Can you work these out from the model? Positions are in its coordinate system, mm. Face numbers are marked on the shaded views. A direction names the side the tool comes from. Give positions to 0.01 mm unless a question says otherwise; leave off trailing zeros. Loops run counter-clockwise (first coordinate to the right, second up) from the corner with the lowest first, then second, coordinate; pieces in that order, holes last. Notation, with made-up numbers: M -14.5,4.5 L 40.5,4.5 A21 cw 40.5,14.5 Z; hole C -37.5,1 d2. An arc over 180 degrees is marked long. Put each result on its own line as item: value. Start each with the question number.
1) If we mould it in two halves opening along Z, with no side actions, what happens to the marked faces 3, 4 and 5? For each: +Z half, -Z half, draft (parallel to the pull), parting line (faces both ways), or undercut.
2) Imagine slicing it at B-B (x = 0). Write out the boundary of the cut face in (y, z), then the cut area to 3 significant figures.
3) For the marked faces 1 and 2, which set-ups out of +Z, -Z, +X, -X, +Y, -Y let a thin tool reach every point of the face, with its end or its side?
4) For P1, Ø8, axis at y = 16, z = -21, coming from the +X side; P2, Ø2, axis at x = 3, y = -0.5, coming from the +Z side; P3, Ø1.5, axis at y = -3.5, z = 9.5, coming from the -X side; P4, Ø5, axis at y = 17.5, z = 12.5, coming from the -X side, each with a flat end and sliding along its axis, tell me the tip position at first contact or that it passes through.
5) Imagine slicing it at A-A (z = 0). Write out the boundary of the cut face in (x, y).
6) Imagine slicing it at D-D (z = 25.5). Write out the boundary of the cut face in (x, y), then the cut area to 3 significant figures.
7) Please list where these lines run through material, in increasing order: line 1 along X through (y, z) = (8, 0); line 2 along X through (y, z) = (-5, 0.5); line 3 along Y through (x, z) = (-94, 11). Write a range as from..to.
8) Imagine slicing it at C-C (y = -6.5). Write out the boundary of the cut face in (x, z), then the cut area to 3 significant figures.
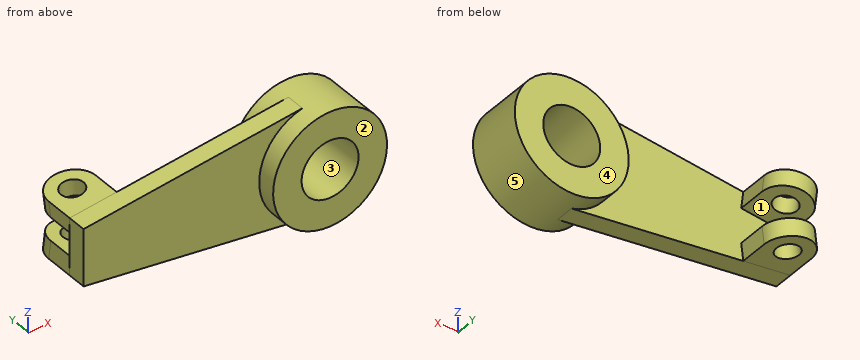
from build123d import *

# Parameters (mm, degrees)
HUB_PROFILE_SKETCH_R   = 30
HUB_60_DEPTH           = 20
LEVER_ARM_DEPTH        = 10
HUB_START              = 20
HUB_EXTENSION_SKETCH_R = 30
HUB_EXTENSION_DEPTH    = 20
CLEVIS_LUG_SKETCH_R    = 6
CLEVIS_LUG_DEPTH       = 9
HUB_RECESS_SKETCH_R    = 30
HUB_RECESS_CUT_DEPTH   = 10
BORE_SKETCH_R          = 15
HUB_BORE_30_DEPTH      = 46


with BuildPart() as part:
    # Hub Profile Sketch → Hub Ø60 (new body)
    with BuildSketch(Plane(origin=(0, 0, 0), x_dir=(1, 0, 0), z_dir=(0, 1, 0))):
        with Locations(Location((0, 0, 0), (0, 0, 270))):
            Circle(HUB_PROFILE_SKETCH_R)
    extrude(amount=HUB_60_DEPTH)

    # Arm Profile Sketch → Lever Arm (add)
    with BuildSketch(Plane(origin=(0, 0, 0), x_dir=(1, 0, 0), z_dir=(0, 1, 0))):
        with BuildLine():
            Line((-122.5, 0), (-30, 0))
            ThreePointArc((-30, 0), (-23.63421499, 18.477658992), (-7.238407879, 29.113664341))
            Line((-7.238407879, 29.113664341), (-122.5, 15))
            Line((-122.5, 15), (-122.5, 0))
        make_face()
        with BuildLine():
            ThreePointArc((-7.238407879, -29.113664341), (-23.63421499, -18.477658992), (-30, 0))
            Line((-30, 0), (-122.5, 0))
            Line((-122.5, 0), (-122.5, -15))
            Line((-122.5, -15), (-7.238407879, -29.113664341))
        make_face()
    extrude(amount=LEVER_ARM_DEPTH)

    # Hub Extension Sketch → Hub Extension (add)
    with BuildSketch(Plane.XZ.offset(HUB_START)):
        with Locations(Location((0, 0, 0), (0, 0, 270))):
            Circle(HUB_EXTENSION_SKETCH_R)
    extrude(amount=-HUB_EXTENSION_DEPTH)

    # Clevis Lug Sketch → Clevis Lug (add)
    with BuildSketch(Plane(origin=(-3.619203939, 0, -29.556832171), x_dir=(-0.9925863886954069, 0, 0.12154119045249893), z_dir=(-0.12154119045249893, 0, -0.9925863886954069))):
        with BuildLine():
            Line((119.768714758, 0), (119.768714758, 25))
            ThreePointArc((119.768714758, 25), (107.268714758, 37.5), (94.768714758, 25))
            Line((94.768714758, 25), (94.768714758, 0))
            Line((94.768714758, 0), (119.768714758, 0))
        make_face()
        with Locations((107.268714758, 25)):
            Circle(CLEVIS_LUG_SKETCH_R, mode=Mode.SUBTRACT)
    extrude(amount=-CLEVIS_LUG_DEPTH)

    # Clevis Lug Mirror: part across plane


with BuildPart() as part_1:
    add(part.part)
    add(part.part.mirror(Plane.XY))

    # Hub Recess Sketch → Hub Recess Cut (cut)
    with BuildSketch(Plane(origin=(0, -20, 0), x_dir=(-1, 0, 0), z_dir=(0, -1, 0))):
        with Locations(Location((0, 0, 0), (0, 0, 90))):
            Circle(HUB_RECESS_SKETCH_R)
    extrude(amount=-HUB_RECESS_CUT_DEPTH, mode=Mode.SUBTRACT)

    # Bore Sketch → Hub Bore Ø30 (cut)
    with BuildSketch(Plane(origin=(0, -10, 0), x_dir=(-1, 0, 0), z_dir=(0, -1, 0))):
        with Locations(Location((0, 0, 0), (0, 0, 90))):
            Circle(BORE_SKETCH_R)
    extrude(amount=-HUB_BORE_30_DEPTH, mode=Mode.SUBTRACT)


solid = part_1.part
Recorded:
1. face 3: undercut
1. face 4: draft
1. face 5: parting line
2. outline: M -10,-30 L 20,-30 L 20,-15 L -10,-15 Z; M -10,15 L 20,15 L 20,30 L -10,30 Z
2. area: 900 mm²
3. face 1: +Y
3. face 2: +Z, -Z, +X, -X, -Y
4. P1: x = 24.72
4. P2: z = 29.93
4. P3: x = -28.7
4. P4: x = -122.5
5. outline: M -122.5,0 L -30,0 L -30,-10 L -15,-10 L -15,20 L -30,20 L -30,10 L -122.5,10 Z; M 15,-10 L 30,-10 L 30,20 L 15,20 Z
6. outline: M -36.75,0 L -15.8,0 L -15.8,-10 L 15.8,-10 L 15.8,20 L -15.8,20 L -15.8,10 L -36.75,10 Z
6. area: 1,160 mm²
7. line 1: -122.5..-15, 15..30
7. line 2: -30..-14.99, 14.99..30
7. line 3: 0..10
8. outline: C 0,0 d60; hole C 0,0 d30
8. area: 2,120 mm²
